```python
from build123d import *

# Parameters (mm, degrees)
GB_T6728_2002_90_X_50_X_4_1_DEPTH = 1550
HOLE_WIZARD_20_0_20_1_D           = 20
PATTERN_LINEAR_1_COUNT            = 6
PATTERN_LINEAR_1_PITCH            = 200
HOLE_WIZARD_14_0_14_2_D           = 14


with BuildPart() as part:
    # Sketch11 → 冷弯空心矩管gb∕t6728-2002 90 X 50 X 4(1) (new body)
    with BuildSketch(Plane(origin=(0, 0, 0), x_dir=(0, 0, 1), z_dir=(1, 0, 0))):
        with BuildLine():
            Line((-19, -45), (19, -45))
            ThreePointArc((19, -45), (23.242640687, -43.242640687), (25, -39))
            Line((25, -39), (25, 39))
            ThreePointArc((25, 39), (23.242640687, 43.242640687), (19, 45))
            Line((19, 45), (-19, 45))
            ThreePointArc((-19, 45), (-23.242640687, 43.242640687), (-25, 39))
            Line((-25, 39), (-25, -39))
            ThreePointArc((-25, -39), (-23.242640687, -43.242640687), (-19, -45))
        make_face()
        with BuildLine():
            Line((-19, -42), (19, -42))
            ThreePointArc((19, -42), (21.121320344, -41.121320344), (22, -39))
            Line((22, -39), (22, 39))
            ThreePointArc((22, 39), (21.121320344, 41.121320344), (19, 42))
            Line((19, 42), (-19, 42))
            ThreePointArc((-19, 42), (-21.121320344, 41.121320344), (-22, 39))
            Line((-22, 39), (-22, -39))
            ThreePointArc((-22, -39), (-21.121320344, -41.121320344), (-19, -42))
        make_face(mode=Mode.SUBTRACT)
    extrude(amount=GB_T6728_2002_90_X_50_X_4_1_DEPTH)

    # Split Bodies 1
    split(bisect_by=Plane(origin=(21.143083968, -30.195453225, 0), x_dir=(-0.819152044288993, -0.5735764363510444, 0), z_dir=(0.5735764363510444, -0.819152044288993, -2.99158375078423e-15)), keep=Keep.TOP)

    # Ø20.0 (20) 直径孔1 (through all)
    with Locations(Plane.XY.offset(25)):
        with Locations((368.533320607, 0)):
            hole_wizard_20_0_20_1 = Hole(HOLE_WIZARD_20_0_20_1_D / 2)

    # 阵列(线性)1: Ø20.0 (20) 直径孔1 ×6
    with Locations(*[(i * PATTERN_LINEAR_1_PITCH, 0, 0) for i in range(1, PATTERN_LINEAR_1_COUNT)]):
        add(hole_wizard_20_0_20_1, mode=Mode.SUBTRACT)

    # Ø14.0 (14) 直径孔2 (through all)
    with Locations(Plane.XY.offset(25)):
        with Locations((115.028466248, 11.128307401), (74.070864034, -17.550514417)):
            Hole(HOLE_WIZARD_14_0_14_2_D / 2)


solid = part.part
```
Geometry: final body of the model. Coordinates: model frame, mm. A direction names the side the tool comes from. Round coordinates to 2 decimals unless told otherwise and drop trailing zeros. Order: outer loops, then holes, each group sorted by start corner. A loop starts at its lowest first (then second) coordinate and runs counter-clockwise, first axis right, second up. Notation, with made-up numbers: (31.5, 0) - (63.5, 0) arc R7 ccw to (63.5, 6) - close; hole circle Ø11 at (-22.5, -3). An arc over 180 degrees is marked (long way). Use CSV: the item, a comma, the result in double quotes. Start each with the question number.
Q1. Section query B-B (z = 0). Return loops of the section in (x, y).
Q2. Access query for faces 4 (the face through (64.57, 0.21, -22.34)), 5 (the face through (768, -17, 22)). Directions: +Z, -Z, +X, -X, +Y, -Y. A direction counts if a zero-diameter tool reaches every point of the face in a straight line with its end or side. Return the directions, or none.
Q3. Mould query, pull axis Y, two halves, no side actions, for faces 1 (the face through (766, -42, 0)), 2 (the face through (764, -45, 0)), 3 (the face through (768, -18, -25)). Classes: +Y half, -Y half, draft (parallel to the pull), parting line (faces both ways), or undercut.
Q4. Section query A-A (x = 1451). Return loops of the section in (y, z).
Q5. Material intervals for line 1 along Z through (x, y) = (873.5, -33.5); line 2 along Y through (x, z) = (755.5, -13.5); line 3 along Z through (x, y) = (702.5, 40), sorted ascending. Write a range as from..to.
Result set:
1,outline,"(0, -45) - (1550, -45) - (1550, -42) - (4.28, -42) - close; (124.25, 42) - (1550, 42) - (1550, 45) - (128.53, 45) - close"
2,face 4,"+Z, -Z, -X, +Y"
2,face 5,"+X, -X"
3,face 1,"undercut"
3,face 2,"-Y half"
3,face 3,"draft"
4,outline,"(-45, -19) arc R6 ccw to (-39, -25) - (39, -25) arc R6 ccw to (45, -19) - (45, 19) arc R6 ccw to (39, 25) - (-39, 25) arc R6 ccw to (-45, 19) - close; hole (-42, -19) arc R3 ccw to (-39, -22) - (39, -22) arc R3 ccw to (42, -19) - (42, 19) arc R3 ccw to (39, 22) - (-39, 22) arc R3 ccw to (-42, 19) - close"
5,line 1,"z = -25..-22, 22..25"
5,line 2,"y = -45..-42, 42..45"
5,line 3,"z = -24.92..-21.83, 21.83..24.92"
